The listing builds one solid part. Answer for the finished solid, in the listing's coordinates (mm). A direction names the side the tool comes from. Give positions to 0.01 mm unless a question says otherwise; leave off trailing zeros. Order: outer loops, then holes, each group sorted by start corner. A loop starts at its lowest first (then second) coordinate and runs counter-clockwise, first axis right, second up. Notation, with made-up numbers: M 81,-18.5 L 127,-18.5 A23 cw 127,-4.5 Z; hole C 42,-22.5 d1. An arc over 180 degrees is marked long. Answer as a JSON object with one key per item and string values. Group by question number.
```python
from build123d import *

# Parameters (mm, degrees)
SKETCH_1_W                   = 50
SKETCH_1_H                   = 9
EXTRUDE_1_DEPTH              = 6
CHAMFER_1_SIZE               = 0.5
HOLE_WIZARD_M3_1_D           = 3.4
HOLE_WIZARD_M3_1_CBORE_D     = 6.5
HOLE_WIZARD_M3_1_CBORE_DEPTH = 4


with BuildPart() as part:
    # 草图1 → 凸台-拉伸1 (new body)
    with BuildSketch(Plane(origin=(0, 0, 0), x_dir=(1, 0, 0), z_dir=(0, 1, 0))):
        Rectangle(SKETCH_1_W, SKETCH_1_H)
    extrude(amount=EXTRUDE_1_DEPTH)

    # 倒角1
    chamfer_1_edges = [part.edges().sort_by_distance(p)[0] for p in [
        (25, 6, 0),
        (0, 6, -4.5),
        (-25, 6, 0),
        (0, 0, -4.5),
        (25, 0, 0),
        (0, 0, 4.5),
        (-25, 0, 0),
        (-25, 3, -4.5),
        (25, 3, -4.5),
        (25, 3, 4.5),
        (-25, 3, 4.5),
        (0, 6, 4.5),
    ]]
    chamfer(chamfer_1_edges, length=CHAMFER_1_SIZE)

    # M3 六角凹头螺钉的柱形沉头孔1 (through all)
    with Locations(Plane(origin=(0, 6, 0), x_dir=(1, 0, 0), z_dir=(0, 1, 0))):
        with Locations((-15, 0), (15, 0)):
            CounterBoreHole(HOLE_WIZARD_M3_1_D / 2, HOLE_WIZARD_M3_1_CBORE_D / 2, HOLE_WIZARD_M3_1_CBORE_DEPTH)


solid = part.part
```
Item 1: Section A-A (y = 3.5) is taken. Determine the outline of the cut face in (x, z), and give its area (3 significant figures).
Item 2: A flat-ended cylindrical pin translates along its axis: P1, Ø2, axis at x = 16.5, z = 0, coming from the +Y side. Find the tip coordinate at first contact, or state that the pin passes through.
Item 3: Section C-C (x = -15) is taken. Determine the outline of the cut face in (y, z), and give its area (3 significant figures).
Item 4: Section D-D (x = 14) is taken. Determine the outline of the cut face in (y, z).
Item 5: Section B-B (z = 0) is taken. Determine the outline of the cut face in (x, y).
Item 6: Determine the mould class of faces 1 (the flat face through (0, 6, 0)), 2 (the flat face through (16.4, 2, 1.4)), 3 (the flat face through (25, 3, 0)) for opening direction X: released by +X, released by -X, zero draft, split by the parting line, or undercut.
Item 7: A tool of negligible diameter and unlimited length cuts with its end or side. For faces 4 (the cylindrical face through (11.753, 4.028, -0.143)), 5 (the flat face through (-25, 3, 0)), from which of +Z, -Z, +X, -X, +Y, -Y can it reach the whole face along a straight path? Write none if from no direction.
Item 8: Consider probe 1 along X at (y, z) = (2.75, -0.5); probe 2 along X at (y, z) = (5, 2); probe 3 along Z at (x, y) = (-15, 3.9). Determine where each line is inside the solid, lowest interval first. Write a range as from..to.
Values found:
{
 "1": {"outline": "M -25,-4 L -24.5,-4.5 L 24.5,-4.5 L 25,-4 L 25,4 L 24.5,4.5 L -24.5,4.5 L -25,4 Z; hole C -15,0 d6.5; hole C 15,0 d6.5", "area": "383 mm^2"},
 "2": {"P1": "stops at y = 2"},
 "3": {"outline": "M 0,-4 L 0.5,-4.5 L 5.5,-4.5 L 6,-4 L 6,-3.25 L 2,-3.25 L 2,-1.7 L 0,-1.7 Z; M 0,1.7 L 2,1.7 L 2,3.25 L 6,3.25 L 6,4 L 5.5,4.5 L 0.5,4.5 L 0,4 Z", "area": "20.7 mm^2"},
 "4": {"outline": "M 0,-4 L 0.5,-4.5 L 5.5,-4.5 L 6,-4 L 6,-3.09 L 2,-3.09 L 2,-1.37 L 0,-1.37 Z; M 0,1.37 L 2,1.37 L 2,3.09 L 6,3.09 L 6,4 L 5.5,4.5 L 0.5,4.5 L 0,4 Z"},
 "5": {"outline": "M -25,0.5 L -24.5,0 L -16.7,0 L -16.7,2 L -18.25,2 L -18.25,6 L -24.5,6 L -25,5.5 Z; M -13.3,0 L 13.3,0 L 13.3,2 L 11.75,2 L 11.75,6 L -11.75,6 L -11.75,2 L -13.3,2 Z; M 16.7,0 L 24.5,0 L 25,0.5 L 25,5.5 L 24.5,6 L 18.25,6 L 18.25,2 L 16.7,2 Z"},
 "6": {"face 1": "zero draft", "face 2": "undercut", "face 3": "released by +X"},
 "7": {"face 4": "+Y", "face 5": "+Z, -Z, -X, +Y, -Y"},
 "8": {"probe 1": "x = -25..-18.21, -11.79..11.79, 18.21..25", "probe 2": "x = -25..-17.56, -12.44..12.44, 17.56..25", "probe 3": "z = -4.5..-3.25, 3.25..4.5"}
}
